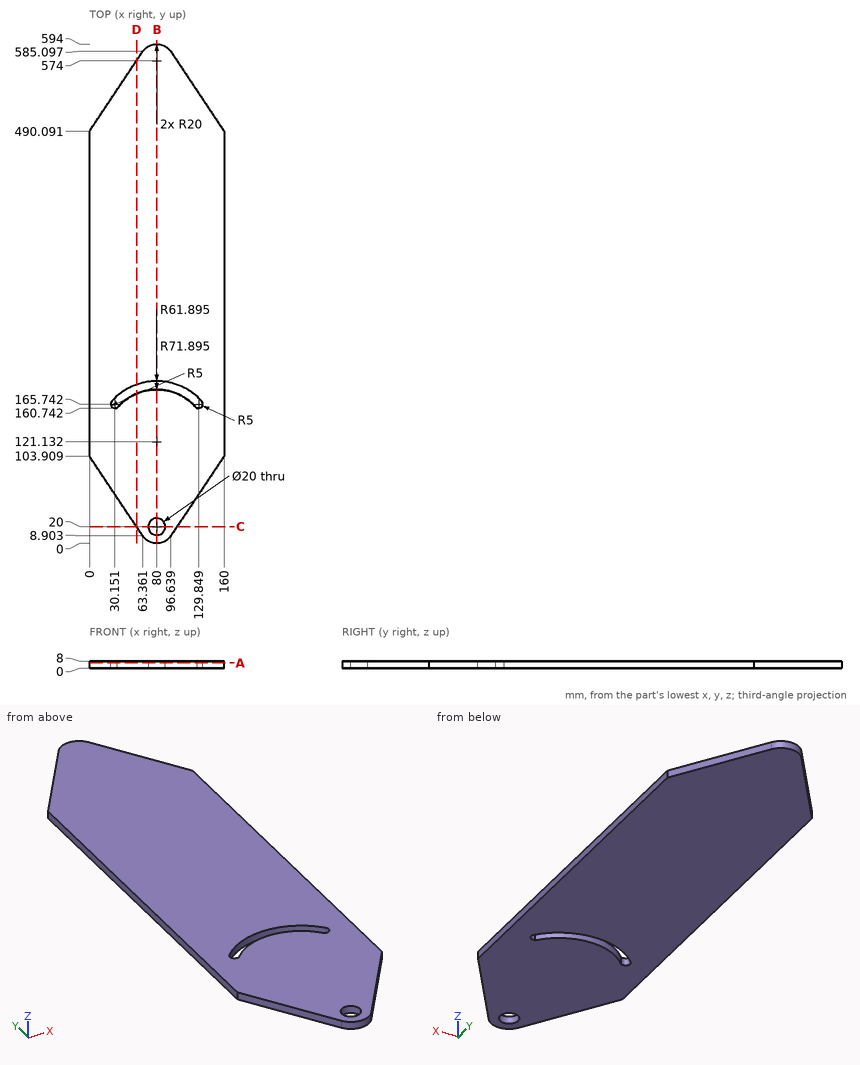
Geometry: see drawing. Coordinates: mm, zero at the bounding-box minimum. Give positions to 0.01 mm unless a question says otherwise; leave off trailing zeros. Loops run counter-clockwise (first coordinate to the right, second up) from the corner with the lowest first, then second, coordinate; pieces in that order, holes last. Notation, with made-up numbers: (22, 84) -> (47, 84) arc R20 ccw to (47, 121) -> close; hole circle Ø5 at (6.5, -5). An arc over 180 degrees is marked (long way). Answer as a JSON object with one key per item and string values. Group by question number.
Item 1: Cut plane A-A, the plane z = 6.25. State how many separate pieces and enclosed holes the cut face has, and give its area (4 significant figures).
Item 2: Cut plane C-C, the plane y = 20. Return the cut outline in (x, z).
Item 3: Cut plane B-B, the plane x = 80. Return the cut outline in (y, z), and give its area (3 significant figures).
Item 4: Cut plane D-D, the plane x = 56. Return the cut outline in (y, z) (1 decimal).
Item 5: Line query: probe 1 along Y at (x, z) = (80, 6.75); probe 2 along X at (y, z) = (20, 5); probe 3 along X at (y, z) = (176.5, 3.5) (1 decimal). Output: solid intervals per line, ascending.
Item 6: Pin query (flat end, axial travel): P1, Ø0.7, axis at x = 128.5, z = 4.5, coming from the +Y side; P2, Ø1, axis at x = 141, z = 1, coming from the -Y side; P3, Ø1.1, axis at x = 31, z = 4, coming from the +Y side. Return the tip coordinate at first contact, or that it passes through.
Checks:
{
 "1": {"separate pieces": "1", "enclosed holes": "2", "area": "79,050 mm²"},
 "2": {"outline": "(55.96, 0) -> (70, 0) -> (70, 8) -> (55.96, 8) -> close; (90, 0) -> (104.04, 0) -> (104.04, 8) -> (90, 8) -> close"},
 "3": {"outline": "(0, 0) -> (10, 0) -> (10, 8) -> (0, 8) -> close; (30, 0) -> (183.03, 0) -> (183.03, 8) -> (30, 8) -> close; (193.03, 0) -> (594, 0) -> (594, 8) -> (193.03, 8) -> close", "area": "4,510 mm²"},
 "4": {"outline": "(19.9, 0) -> (178.2, 0) -> (178.2, 8) -> (19.9, 8) -> close; (188.9, 0) -> (574.1, 0) -> (574.1, 8) -> (188.9, 8) -> close"},
 "5": {"probe 1": "y = 0 to 10, 30 to 183.03, 193.03 to 594", "probe 2": "x = 55.96 to 70, 90 to 104.04", "probe 3": "x = 0 to 34.1, 52.3 to 107.7, 125.9 to 160"},
 "6": {"P1": "stops at y = 537.85", "P2": "stops at y = 74.67", "P3": "stops at y = 537.4"}
}
